```python
from build123d import *

# Parameters (mm, degrees)
SKETCH1_R               = 203.294925519
SKETCH1_R_2             = 173.294925519
BOSS_EXTRUDE1_DEPTH     = 10
CUT_EXTRUDE1_START      = -185
CUT_EXTRUDE1_DEPTH      = 185
CUT_EXTRUDE2_DEPTH      = 185
CUT_EXTRUDE3_DEPTH      = 484.877792972
CUT_EXTRUDE3_DEPTH_BACK = 484.877792972
SKETCH5_R               = 4


with BuildPart() as part:
    # Sketch1 → Boss-Extrude1 (new body)
    with BuildSketch(Plane.XY):
        with Locations((291.585214163, 182.730697222)):
            Circle(SKETCH1_R)
        with Locations((291.585214163, 182.730697222)):
            Circle(SKETCH1_R_2, mode=Mode.SUBTRACT)
    extrude(amount=-BOSS_EXTRUDE1_DEPTH)

    # Sketch2 → Cut-Extrude1 (cut)
    with BuildSketch(Plane(origin=(0, 0, -10), x_dir=(-1, 0, 0), z_dir=(0, 0, -1)).offset(CUT_EXTRUDE1_START)):
        with BuildLine():
            Line((-291.585214163, 9.435771703), (-291.585214163, -33.905509081))
            ThreePointArc((-291.585214163, -33.905509081), (-508.221420466, 182.730697222), (-291.585214163, 399.366903525))
            Line((-291.585214163, 399.366903525), (-291.585214163, 356.025622742))
            ThreePointArc((-291.585214163, 356.025622742), (-464.880139683, 182.730697222), (-291.585214163, 9.435771703))
        make_face()
    extrude(amount=CUT_EXTRUDE1_DEPTH, mode=Mode.SUBTRACT)

    # Sketch3 → Cut-Extrude2 (cut)
    with BuildSketch(Plane(origin=(0, 0, -10), x_dir=(-1, 0, 0), z_dir=(0, 0, -1))):
        with BuildLine():
            ThreePointArc((-228.398227799, 1.480100191), (-145.149611461, 58.629978323), (-102.426094867, 150.123922508))
            ThreePointArc((-102.426094867, 150.123922508), (-105.727828311, 154.801028245), (-110.404934048, 151.499294801))
            ThreePointArc((-110.404934048, 151.499294801), (-151.326348425, 63.864617192), (-231.063490803, 9.125353407))
            ThreePointArc((-231.063490803, 9.125353407), (-233.553485909, 3.970095297), (-228.398227799, 1.480100191))
        make_face()
    extrude(amount=-CUT_EXTRUDE2_DEPTH, mode=Mode.SUBTRACT)

    # Sketch5 → Cut-Extrude3 (cut, two sides: drawn at the far end of the back side and taken through both)
    with BuildSketch(Plane.XY.offset(-CUT_EXTRUDE3_DEPTH_BACK)):
        with Locations((233.317748738, 361.783430933)):
            Circle(SKETCH5_R)
        with Locations((203.411601384, 349.104953001)):
            Circle(SKETCH5_R)
        with Locations((162.898022452, 320.188274917)):
            Circle(SKETCH5_R)
    extrude(amount=CUT_EXTRUDE3_DEPTH + CUT_EXTRUDE3_DEPTH_BACK, mode=Mode.SUBTRACT)


solid = part.part
```
Check sheet for the modelled part. Datum: model origin and axes. Units: mm. A direction names the side the tool comes from. Give positions to 0.01 mm unless a question says otherwise; leave off trailing zeros. Order: outer loops, then holes, each group sorted by start corner. A loop starts at its lowest first (then second) coordinate and runs counter-clockwise, first axis right, second up. Notation, with made-up numbers: M -19,-9 L -15,-9 A10 ccw -15,-5 Z; hole C 62,26.25 d6. An arc over 180 degrees is marked long. Answer in a Markdown table with one row per item.
1) Cross-section at B-B, the plane y = 113.5. Enter the section's corners in (x, z).
Filled sheet:
| item | result |
|---|---|
| outline | M 100.44,-10 L 112.56,-10 L 112.56,0 L 100.44,0 Z; M 121.27,-10 L 132.72,-10 L 132.72,0 L 121.27,0 Z |
2) Cross-section at A-A, the plane x = 264. Enter the section's corners in (y, z), plus the area to 3 significant figures.
Filled sheet:
| item | result |
|---|---|
| outline | M -18.68,-10 L 11.65,-10 L 11.65,0 L -18.68,0 Z; M 353.82,-10 L 384.15,-10 L 384.15,0 L 353.82,0 Z |
| area | 607 mm2 |
3) Gauge pin test, flat ends, axial feed: P1, Ø4, axis at y = 329, z = -2, coming from the +X side; P2, Ø10.5, axis at x = 233.32, y = 361.78, coming from the -Z side; P3, Ø3, axis at x = 131.5, z = -2.5, coming from the -Y side; P4, Ø4, axis at y = 220, z = -5.5, coming from the -X side. Record the tip position at first contact, or that the pin passes through.
Filled sheet:
| item | result |
|---|---|
| P1 | stops at x = 201.88 |
| P2 | stops at z = -10 |
| P3 | stops at y = 55.53 |
| P4 | stops at x = 91.37 |
4) Cross-section at D-D, the plane z = -5.25. Enter the section's corners in (x, y), plus the area to 3 significant figures.
Filled sheet:
| item | result |
|---|---|
| outline | M 291.59,-20.56 L 291.59,9.44 A173.29 cw 291.59,356.03 L 291.59,386.03 A203.29 ccw Z; hole M 102.43,150.12 A191.95 ccw 228.4,1.48 A4.05 ccw 231.06,9.13 A183.85 cw 110.4,151.5 A4.05 ccw Z; hole C 162.9,320.19 d8; hole C 203.41,349.1 d8; hole C 233.32,361.78 d8 |
| area | 15,900 mm2 |
5) Thickness scan on L1, parallel to Y at x = 147, z = -7.25; L2, parallel to Y at x = 216.5, z = -6.25; L3, parallel to Y at x = 269, z = -9.5. Record the ranges inside material, lowest first. Write a range as [from, to].
Filled sheet:
| item | result |
|---|---|
| L1 | y = [39.82, 56.48], [69.17, 87.2], [278.26, 325.64] |
| L2 | y = [-6.19, 6.08], [14.91, 26.55], [338.91, 371.65] |
| L3 | y = [-19.31, 10.91], [354.55, 384.77] |
6) Access from +Z, -Z, +X, -X, +Y, -Y to the whole of each face (thin tool, end or side, straight path). Record for faces 5 (the cylindrical face through (146.08, 57.54, -5.07)), 6 (the flat face through (114, 199, -10)).
Filled sheet:
| item | result |
|---|---|
| face 5 | +Z, -Z |
| face 6 | -Z, +X, -X, +Y, -Y |
7) Release check for a two-part mould opening along X. For faces 1 (the cylindrical face through (150.444, 64.913, -5.07)), 2 (the flat face through (291.585, 371, -5)), 3 (the flat face through (114, 199, 0)), 4 (the cylindrical face through (233.58, 4.05, -5.07)) record: +X half, -X half, draft (parallel to the pull), parting line (faces both ways), or undercut.
Filled sheet:
| item | result |
|---|---|
| face 1 | undercut |
| face 2 | +X half |
| face 3 | draft |
| face 4 | undercut |
8) Cross-section at C-C, the plane x = 193. Enter the section's corners in (y, z), plus the area to 3 significant figures.
Filled sheet:
| item | result |
|---|---|
| outline | M 4.94,-10 L 18.03,-10 L 18.03,0 L 4.94,0 Z; M 27.54,-10 L 40.21,-10 L 40.21,0 L 27.54,0 Z; M 325.25,-10 L 360.52,-10 L 360.52,0 L 325.25,0 Z |
| area | 610 mm2 |
